Part print with two shaded views. Sizes in mm from the minimum x, y, z corner. Give positions to 0.01 mm unless a question says otherwise; leave off trailing zeros. Order: outer loops, then holes, each group sorted by start corner. A loop starts at its lowest first (then second) coordinate and runs counter-clockwise, first axis right, second up. Notation, with made-up numbers: (58, 9.5) -> (69, 9.5) arc R10 ccw to (69, 28.5) -> close; hole circle Ø2 at (8, 6.25). An arc over 180 degrees is marked (long way). Answer as CSV lines item,"result".
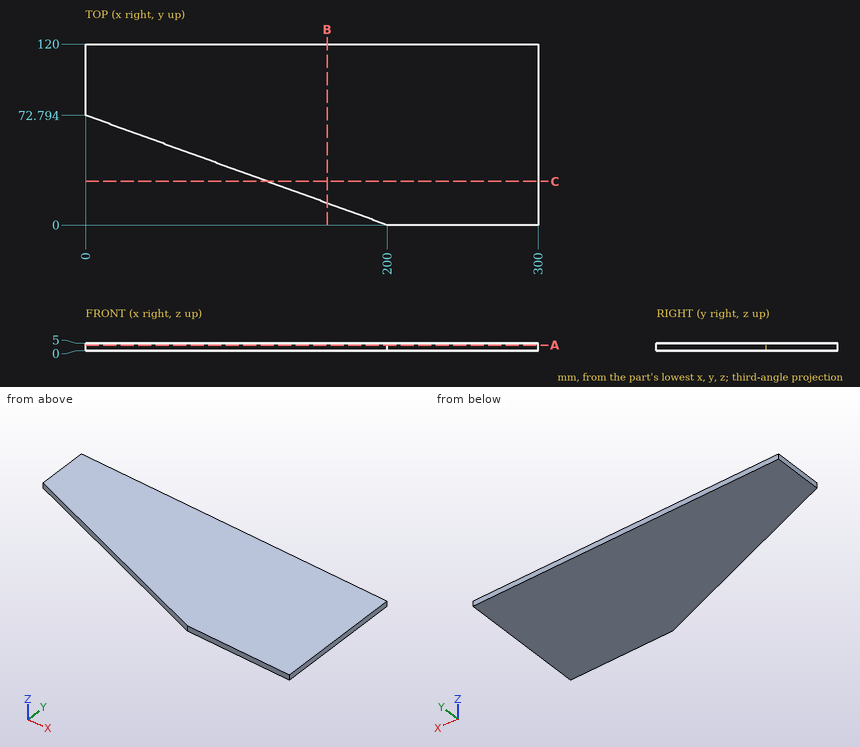
1) Band-saw the part on A-A, the plane z = 3.75. Write the cut outline in (x, y), then the cut area to 3 significant figures.
Data:
outline,"(0, 72.79) -> (200, 0) -> (300, 0) -> (300, 120) -> (0, 120) -> close"
area,"28,700 mm2"
2) Band-saw the part on B-B, the plane x = 160. Write the cut outline in (y, z), then the cut area to 3 significant figures.
Data:
outline,"(14.56, 0) -> (120, 0) -> (120, 5) -> (14.56, 5) -> close"
area,"527 mm2"
3) Band-saw the part on C-C, the plane y = 29. Write the cut outline in (x, z).
Data:
outline,"(120.32, 0) -> (300, 0) -> (300, 5) -> (120.32, 5) -> close"
4) Wall check: line 1 along Y through (x, z) = (40.5, 0.6); line 2 along Y through (x, z) = (24.5, 2.25). Give the ranges that are in metal, low to high. Write a range as [from, to].
Data:
line 1,"y = [58.05, 120]"
line 2,"y = [63.88, 120]"
5) Pin check, flat tip, straight feed: P1, Ø6, axis at x = 124.5, y = 101.5, coming from the -Z side. Stop position of the tip, or through.
Data:
P1,"stops at z = 0"
